from build123d import *

# Parameters (mm, degrees)
BASE_BLOCK_63MM_DEPTH      = 63
PROFILE_CUT_63MM_DEPTH     = 63
SIDE_BOSS_SKETCH_W         = 63
SIDE_BOSS_SKETCH_H         = 90
SIDE_BOSS_16MM_DEPTH       = 16
STEP_CUT_21MM_DEPTH        = 21
CURVED_END_BOSS_21MM_DEPTH = 21
POCKET_CUT_SKETCH_W        = 21
POCKET_CUT_SKETCH_H        = 17.5
POCKET_CUT_40MM_DEPTH      = 40
HOLE_A_SKETCH_W            = 73
HOLE_A_SKETCH_H            = 42
HOLE_A_17_5MM_DEEP_DEPTH   = 17.5
HOLE_B_SKETCH_W            = 73
HOLE_B_SKETCH_H            = 42
HOLE_B_17_5MM_DEEP_DEPTH   = 17.5
END_CUT_SKETCH_R           = 11
END_CUT_SKETCH_R_2         = 8
END_CUT_SKETCH_R_3         = 5
END_CUT_30MM_DEPTH         = 30


with BuildPart() as part:
    # Base Profile Sketch → Base Block 63mm (new body)
    with BuildSketch(Plane.XY):
        Polygon((0, 0), (115, 0), (115, 90), (54, 90), (22, 90), (-4, 90), (-4, 0), align=None)
    extrude(amount=BASE_BLOCK_63MM_DEPTH)

    # Profile Cut Sketch → Profile Cut 63mm (cut)
    with BuildSketch(Plane.XY.offset(63)):
        Polygon((18, 60), (18, 72.5), (18, 90), (-4, 90), (-4, 72.5), (-4, 60), align=None)
        Polygon((18, 30), (-4, 30), (-4, 17.5), (-4, 0), (18, 0), (18, 17.5), align=None)
    extrude(amount=-PROFILE_CUT_63MM_DEPTH, mode=Mode.SUBTRACT)

    # Side Boss Sketch → Side Boss 16mm (add)
    with BuildSketch(Plane(origin=(115, 0, 0), x_dir=(0, 0, -1), z_dir=(1, 0, 0))):
        with Locations((-31.5, 45)):
            Rectangle(SIDE_BOSS_SKETCH_W, SIDE_BOSS_SKETCH_H)
    extrude(amount=SIDE_BOSS_16MM_DEPTH)

    # Step Cut Sketch → Step Cut 21mm (cut)
    with BuildSketch(Plane.XY.offset(63)):
        Polygon((18, 90), (91, 90), (131, 90), (131, 0), (91, 0), (18, 0), (18, 30), (-4, 30), (-4, 60), (18, 60), align=None)
    extrude(amount=-STEP_CUT_21MM_DEPTH, mode=Mode.SUBTRACT)

    # Curved End Boss Sketch → Curved End Boss 21mm (add)
    with BuildSketch(Plane.XY.offset(42)):
        with BuildLine():
            Line((131, 90), (131, 0))
            ThreePointArc((131, 0), (138.429264164, 45), (131, 90))
        make_face()
    extrude(amount=-CURVED_END_BOSS_21MM_DEPTH)

    # Pocket Cut Sketch → Pocket Cut 40mm (cut)
    with BuildSketch(Plane(origin=(131, 0, 0), x_dir=(0, 0, -1), z_dir=(1, 0, 0))):
        with Locations((-10.5, 81.25)):
            Rectangle(POCKET_CUT_SKETCH_W, POCKET_CUT_SKETCH_H)
        with Locations((-10.5, 8.75)):
            Rectangle(POCKET_CUT_SKETCH_W, POCKET_CUT_SKETCH_H)
    extrude(amount=-POCKET_CUT_40MM_DEPTH, mode=Mode.SUBTRACT)

    # Hole A Sketch → Hole A 17.5mm Deep (cut)
    with BuildSketch(Plane.XZ):
        with Locations((54.5, 21)):
            Rectangle(HOLE_A_SKETCH_W, HOLE_A_SKETCH_H)
    extrude(amount=-HOLE_A_17_5MM_DEEP_DEPTH, mode=Mode.SUBTRACT)

    # Hole B Sketch → Hole B 17.5mm Deep (cut)
    with BuildSketch(Plane(origin=(0, 90, 0), x_dir=(1, 0, 0), z_dir=(0, 1, 0))):
        with Locations((54.5, -21)):
            Rectangle(HOLE_B_SKETCH_W, HOLE_B_SKETCH_H)
    extrude(amount=-HOLE_B_17_5MM_DEEP_DEPTH, mode=Mode.SUBTRACT)

    # End Cut Sketch → End Cut 30mm (cut)
    with BuildSketch(Plane.XY.offset(42)):
        with Locations((111, 45)):
            Circle(END_CUT_SKETCH_R)
        with Locations((70, 45)):
            Circle(END_CUT_SKETCH_R_2)
        with Locations((38, 45)):
            Circle(END_CUT_SKETCH_R_2)
        with Locations((12, 45)):
            Circle(END_CUT_SKETCH_R_3)
    extrude(amount=-END_CUT_30MM_DEPTH, mode=Mode.SUBTRACT)


solid = part.part
The listing builds one solid part. Answer for the finished solid, in the listing's coordinates (mm). A direction names the side the tool comes from. Coordinates: 2 decimals unless noted, no trailing zeros. Order: outer loops, then holes, each group sorted by start corner. A loop starts at its lowest first (then second) coordinate and runs counter-clockwise, first axis right, second up.
Q1. For a pull along X with two mould halves and no side action, classify faces 6 (the face through (63, 45, 0)), 7 (the face through (15, 49, 27)), 8 (the face through (91, 81, 32)) as pulls with the +X half, pulls with the -X half, needs draft (parallel to the pull), parting line crosses it, or undercut.
Q2. Consider line 1 (Y direction, x = 111, z = 33.25); line 2 (X direction, y = 47.5, z = 39); line 3 (X direction, y = 42, z = 22). Determine where each line is inside the solid, lowest interval first.
Q3. Which of the six approach directions +Z, -Z, +X, -X, +Y, -Y give full straight-line access (tool end or side, diameter ignored) to faces 1 (the face through (91, 9, 31)), 2 (the face through (138.428, 44.359, 31.647)), 3 (the face through (131, 45, 11)), 4 (the face through (7, 60, 21)), 5 (the face through (70, 45, 12))?
Q4. A cutting plane is placed at C-C, the plane z = 9.5. Write down the section's boundary in (x, y), and give its area (4 significant figures).
Q5. A cutting plane is placed at D-D, the plane y = 26. Write down the section's boundary in (x, z).
Q6. Given P1, Ø14.5, axis at x = 38, y = 45, coming from the +Z side; P2, Ø1.5, axis at x = 16.5, z = 9.5, coming from the -Y side; P3, Ø12.5, axis at x = 57, z = 26.5, coming from the +Y side, each flat-ended and moving along its own axis, determine where each tip first touches the part or whether it passes through.
Q7. A cutting plane is placed at B-B, the plane x = 12. Write down the section's boundary in (y, z).
Q8. A cutting plane is placed at A-A, the plane z = 37.5. Write down the section's boundary in (x, y).
Answers follow:
1. face 6: needs draft
1. face 7: undercut
1. face 8: pulls with the -X half
2. line 1: y = 0 to 34, 56 to 90
2. line 2: x = -4 to 7.67, 16.33 to 30.4, 45.6 to 62.4, 77.6 to 100.29, 121.71 to 138.41
2. line 3: x = -4 to 8, 16 to 30.58, 45.42 to 62.58, 77.42 to 100.42, 121.58 to 138.4
3. face 1: +Z, -Z, -X, -Y
3. face 2: +Z, -Z, +X
3. face 3: -Z, +X, +Y, -Y
3. face 4: +Z, -Z, -X, +Y
3. face 5: +Z
4. outline: (-4, 30) - (18, 30) - (18, 17.5) - (131, 17.5) - (131, 72.5) - (18, 72.5) - (18, 60) - (-4, 60) - close
4. area: 6,875 mm2
5. outline: (18, 0) - (131, 0) - (131, 21) - (137.13, 21) - (137.13, 42) - (18, 42) - close
6. P1: stops at z = 12
6. P2: stops at y = 30
6. P3: stops at y = 72.5
7. outline: (30, 0) - (60, 0) - (60, 42) - (50, 42) - (50, 12) - (40, 12) - (40, 42) - (30, 42) - close
8. outline: (-4, 30) - (18, 30) - (18, 17.5) - (91, 17.5) - (91, 0) - (131, 0) arc R140 ccw to (131, 90) - (91, 90) - (91, 72.5) - (18, 72.5) - (18, 60) - (-4, 60) - close; hole circle Ø10 at (12, 45); hole circle Ø16 at (38, 45); hole circle Ø16 at (70, 45); hole circle Ø22 at (111, 45)
